from build123d import *


with BuildPart() as part:
    # Sketch1 → Revolve1 (revolve)
    with BuildSketch(Plane.XZ, mode=Mode.PRIVATE) as revolve1_sk:
        Polygon((19.5, 0), (19.5, 9), (13, 9), (12.5, 8.5), (12.5, -50.5), (13, -51), (17.5, -51), (17.5, 0), align=None)
    revolve(revolve1_sk.sketch.rotate(Axis((0, 0, 9), (0, 0, -1)), 180), axis=Axis((0, 0, 9), (0, 0, -1)))


solid = part.part
Source: CAD feature listing. Evaluate the final solid. Frame: model axes, mm. Round coordinates to 2 decimals unless told otherwise and drop trailing zeros. Write each loop counter-clockwise with the first axis right and the second up, starting at its lowest first coordinate (ties: lowest second). Pieces come first, ordered by that corner, then holes. Notation, with made-up numbers: M 68,-28 L 80,-28 A17 ccw 80,1 Z; hole C 87,-4 d7. An arc over 180 degrees is marked long. One line per item, written item: value. Start each with the question number.
Item 1: Ray query, L1, parallel to Y at x = 0, z = -36.5; L2, parallel to Z at x = -15, y = 9.5; L3, parallel to Y at x = 4.5, z = -40.5. Return the intervals inside material, ascending. Write a range as from..to.
Item 2: Section query C-C (z = -33). Return the cut outline in (x, y), plus the area to 3 significant figures.
Item 3: Pin query (flat end, axial travel): pin 1 (3 mm diameter, centred on x = -12, y = -15.5, fed in from -Z); pin 2 (8 mm diameter, centred on x = 14, z = -33.5, fed in from +Y); pin 3 (4 mm diameter, centred on x = -12.5, y = 0, fed in from +Z); pin 4 (2 mm diameter, centred on y = -7.5, z = -44, fed in from -X). Return the tip coordinate at first contact, or that it passes through.
Item 4: Section query D-D (y = 15.5). Return the cut outline in (x, z).
Item 5: Section query A-A (x = 0). Return the cut outline in (y, z), plus the area to 4 significant figures.
Item 6: Mould query, pull axis X, two halves, no side actions, for faces 1 (the flat face through (-13, 12, 0)), 2 (the cylindrical face through (-11.923, 3.755, -21.413)), 3 (the cylindrical face through (3.794, -17.084, -25.143)). Classes: pulls with the +X half, pulls with the -X half, needs draft (parallel to the pull), parting line crosses it, or undercut.
Result set:
1. L1: y = -17.5..-12.5, 12.5..17.5
1. L2: z = 0..9
1. L3: y = -16.91..-11.66, 11.66..16.91
2. outline: C 0,0 d35; hole C 0,0 d25
2. area: 471 mm²
3. pin 1: stops at z = 0
3. pin 2: stops at y = 14.36
3. pin 3: stops at z = 9
3. pin 4: stops at x = -16.25
4. outline: M -11.83,0 L -8.12,0 L -8.12,-51 L 8.12,-51 L 8.12,0 L 11.83,0 L 11.83,9 L -11.83,9 Z
5. outline: M -19.5,0 L -17.5,0 L -17.5,-51 L -13,-51 L -12.5,-50.5 L -12.5,8.5 L -13,9 L -19.5,9 Z; M 12.5,-50.5 L 13,-51 L 17.5,-51 L 17.5,0 L 19.5,0 L 19.5,9 L 13,9 L 12.5,8.5 Z
5. area: 635.5 mm²
6. face 1: needs draft
6. face 2: undercut
6. face 3: parting line crosses it
